from build123d import *

# Parameters (mm, degrees)
SKETCH1_R             = 10
BOSS_EXTRUDE1_DEPTH   = 100
M8_TAPPED_HOLE1_D     = 6.8
M8_TAPPED_HOLE1_DEPTH = 22.25
M8_TAPPED_HOLE1_TIP   = 2.042926105
CHAMFER1_SIZE         = 1
CHAMFER3_SIZE         = 1
M8_TAPPED_HOLE2_D     = 6.8
M8_TAPPED_HOLE2_DEPTH = 22.25
M8_TAPPED_HOLE2_TIP   = 2.042926105


with BuildPart() as part:
    # Sketch1 → Boss-Extrude1 (new body)
    with BuildSketch(Plane.XY):
        Circle(SKETCH1_R)
    extrude(amount=BOSS_EXTRUDE1_DEPTH)

    # M8 Tapped Hole1
    with Locations(Plane.XY.offset(100)):
        with Locations((0, 0)):
            Hole(M8_TAPPED_HOLE1_D / 2, depth=M8_TAPPED_HOLE1_DEPTH)
            with Locations((0, 0, -(M8_TAPPED_HOLE1_DEPTH + M8_TAPPED_HOLE1_TIP / 2))):  # 118° drill point
                Cone(0, M8_TAPPED_HOLE1_D / 2, M8_TAPPED_HOLE1_TIP, mode=Mode.SUBTRACT)

    # Chamfer1
    chamfer1_edges = [part.edges().sort_by_distance(p)[0] for p in [
        (-10, 0, 100),
    ]]
    chamfer(chamfer1_edges, length=CHAMFER1_SIZE)

    # Chamfer3
    chamfer3_edges = [part.edges().sort_by_distance(p)[0] for p in [
        (-10, 0, 0),
    ]]
    chamfer(chamfer3_edges, length=CHAMFER3_SIZE)

    # M8 Tapped Hole2
    with Locations(Plane(origin=(0, 0, 0), x_dir=(-1, 0, 0), z_dir=(0, 0, -1))):
        with Locations((0, 0)):
            Hole(M8_TAPPED_HOLE2_D / 2, depth=M8_TAPPED_HOLE2_DEPTH)
            with Locations((0, 0, -(M8_TAPPED_HOLE2_DEPTH + M8_TAPPED_HOLE2_TIP / 2))):  # 118° drill point
                Cone(0, M8_TAPPED_HOLE2_D / 2, M8_TAPPED_HOLE2_TIP, mode=Mode.SUBTRACT)


solid = part.part
Part model, mm, in its own coordinate system. A direction names the side the tool comes from. Give positions to 0.01 mm unless a question says otherwise; leave off trailing zeros. Loops run counter-clockwise (first coordinate to the right, second up) from the corner with the lowest first, then second, coordinate; pieces in that order, holes last. Notation, with made-up numbers: (-11.5, 89.25) -> (36.5, 89.25) arc R20 cw to (36.5, 105.25) -> close; hole circle Ø6 at (85, -18). An arc over 180 degrees is marked (long way). Write each question's results on one line, items separated by ' | '. Start each with the question number.
Q1. Which spindle directions (+Z, -Z, +X, -X, +Y, -Y) get a long thin tool onto all of the face, cutting with end or side? Do faces 4 (the face through (0.74, -3.32, 88.72)), 5 (the face through (0, -4, 0)), 6 (the face through (-0.74, -3.32, 11.28)). Say none if no direction does.
Q2. Band-saw the part on A-A on z = 16.5. List the corners of the cut face in (x, y), plus the area to 3 significant figures.
Q3. Pin check, flat tips, straight feed: P1, Ø4, axis at y = -8, z = 17.5, coming from the +X side; P2, Ø4, axis at x = -6.5, y = -3.5, coming from the -Z side; P3, Ø12, axis at y = -8, z = 87, coming from the -X side; P4, Ø5.5, axis at x = 0, y = 0, coming from the -Z side. Stop position of each tip, or through.
Q4. Pull direction Y, two halves, no side cores. Call faces 1 (the face through (0, -4, 100)), 2 (the face through (-0.128, -0.576, 76.062)), 3 (the face through (-2.17, -9.76, 49.31)): +Y half, -Y half, draft (parallel to the pull), parting line (faces both ways), or undercut.
Q5. Band-saw the part on B-B on z = 45.5. List the corners of the cut face in (x, y).
Q6. Wall check: L1, parallel to Y at x = 0, z = 15; L2, parallel to X at y = 4.5, z = 58.5; L3, parallel to Y at x = -3.5, z = 35. Give the ranges that are in metal, low to high.
Results are:
1) face 4: +Z | face 5: -Z, +X, -X, +Y, -Y | face 6: -Z
2) outline: circle Ø20 at (0, 0); hole circle Ø6.8 at (0, 0) | area: 278 mm²
3) P1: stops at x = 8 | P2: stops at z = 0 | P3: stops at x = -9.8 | P4: stops at z = 22.64
4) face 1: draft | face 2: undercut | face 3: parting line
5) outline: circle Ø20 at (0, 0)
6) L1: y = -10 to -3.4, 3.4 to 10 | L2: x = -8.93 to 8.93 | L3: y = -9.37 to 9.37
